Source: CAD feature listing. Evaluate the final solid. Frame: model axes, mm. A direction names the side the tool comes from. Coordinates: 2 decimals unless noted, no trailing zeros. Write each loop counter-clockwise with the first axis right and the second up, starting at its lowest first coordinate (ties: lowest second). Pieces come first, ordered by that corner, then holes. Notation, with made-up numbers: (-32.75, 44.5) - (16.25, 44.5) arc R22 cw to (16.25, 67.5) - close; hole circle Ø1 at (20.25, -19). An arc over 180 degrees is marked (long way). One line per item, written item: value.
from build123d import *

# Parameters (mm, degrees)
EXTRUDE_1_DEPTH     = 15
SKETCH_2_R          = 13
CUT_EXTRUDE_2_DEPTH = 10


with BuildPart() as part:
    # 草图1 → 拉伸1 (new, symmetric)
    with BuildSketch(Plane.XY):
        with BuildLine():
            ThreePointArc((-7.220859013, 49.475844562), (-35.355230678, 35.355447441), (-49.47580029, 7.221162349))
            add(Edge.make_bspline(
                [(-49.47580029, -7.221162349), (-36.725591286, 0), (-49.47580029, 7.221162349)],
                knots=[2.665650331, 2.665650331, 2.665650331, 3.617534976, 3.617534976, 3.617534976], degree=2, weights=[1, 0.888861367, 1]))
            ThreePointArc((-49.47580029, -7.221162349), (-35.355230678, -35.355447441), (-7.220859013, -49.475844562))
            add(Edge.make_bspline(
                [(7.220859013, -49.475844562), (0, -36.72563521), (-7.220859013, -49.475844562)],
                knots=[2.665650231, 2.665650231, 2.665650231, 3.617535076, 3.617535076, 3.617535076], degree=2, weights=[1, 0.888861321, 1]))
            ThreePointArc((7.220859013, -49.475844562), (35.063945901, -35.644350154), (49.350641932, -8.032069525))
            add(Edge.make_bspline(
                [(49.350641932, 8.032069525), (36.37710154, 0), (49.350641932, -8.032069525)],
                knots=[5.748433423, 5.748433423, 5.748433423, 6.817937192, 6.817937192, 6.817937192], degree=2, weights=[1, 0.860395102, 1]))
            ThreePointArc((49.350641932, 8.032069525), (35.063945901, 35.644350154), (7.220859013, 49.475844562))
            add(Edge.make_bspline(
                [(-7.220859013, 49.475844562), (0, 36.72563521), (7.220859013, 49.475844562)],
                knots=[2.665650231, 2.665650231, 2.665650231, 3.617535076, 3.617535076, 3.617535076], degree=2, weights=[1, 0.888861321, 1]))
        make_face()
        with BuildLine():
            Line((3, -6.873863542), (3, -12.5))
            Line((3, -12.5), (-3, -12.5))
            Line((-3, -12.5), (-3, -6.873863542))
            ThreePointArc((-3, -6.873863542), (-5.303300859, -5.303300859), (-6.873863542, -3))
            Line((-6.873863542, -3), (-12.5, -3))
            Line((-12.5, -3), (-12.5, 3))
            Line((-12.5, 3), (-6.873863542, 3))
            ThreePointArc((-6.873863542, 3), (-5.303300859, 5.303300859), (-3, 6.873863542))
            Line((-3, 6.873863542), (-3, 12.5))
            Line((-3, 12.5), (3, 12.5))
            Line((3, 12.5), (3, 6.873863542))
            ThreePointArc((3, 6.873863542), (5.303300859, 5.303300859), (6.873863542, 3))
            Line((6.873863542, 3), (12.5, 3))
            Line((12.5, 3), (12.5, -3))
            Line((12.5, -3), (6.873863542, -3))
            ThreePointArc((6.873863542, -3), (5.303300859, -5.303300859), (3, -6.873863542))
        make_face(mode=Mode.SUBTRACT)
    extrude(amount=EXTRUDE_1_DEPTH, both=True)

    # 草图2 → 拉伸2 (cut)
    with BuildSketch(Plane.XY.offset(15)):
        Circle(SKETCH_2_R)
    extrude(amount=-CUT_EXTRUDE_2_DEPTH, mode=Mode.SUBTRACT)


solid = part.part
1) Section query A-A on y = 15. Output: boundary loops of the cut face in (x, z), then the cut area to 3 significant figures.
Values found:
outline: (-47.7, -15) - (47.7, -15) - (47.7, 15) - (-47.7, 15) - close
area: 2,860 mm2
2) Material intervals for line 1 (Y direction, x = 0, z = 10.75); line 2 (X direction, y = 12, z = -4.5); line 3 (X direction, y = 8, z = -13), sorted ascending.
Values found:
line 1: -43.48 to -13, 13 to 43.48
line 2: -48.54 to -3, 3 to 48.54
line 3: -49.36 to -3, 3 to 49.3
3) Contact query for flat-ended pins moving along their axis: P1, Ø21, axis at x = 1, y = 1, coming from the +Z side; P2, Ø3, axis at y = 0, z = -9.5, coming from the +X side; P3, Ø1.5, axis at x = -12, z = 8, coming from the +Y side. Output: stop coordinate, or through.
Values found:
P1: z = 5
P2: x = 43.55
P3: y = 48.72
4) Reachability of faces 1 (the cylindrical face through (-10.316, -7.91, 10.07)), 2 (the flat face through (10, -10, -15)), 3 (the flat face through (3, 10, -5)) from +Z, -Z, +X, -X, +Y, -Y: full face, straight path, thin tool, end or side. Return the list, or none.
Values found:
face 1: +Z
face 2: -Z, +X, -X, +Y, -Y
face 3: +Z, -Z
5) Draft query along Y for faces 4 (the cylindrical face through (34.7, -36, 0.2)), 5 (the cylindrical face through (-35.04, 35.67, 0.21)), 6 (the cylindrical face through (-5.275, -5.331, -4.86)), 7 (the flat face through (-5, 6, 5)). Return one class per face: released by +Y, released by -Y, zero draft, split by the parting line, or undercut.
Values found:
face 4: released by -Y
face 5: released by +Y
face 6: undercut
face 7: undercut
6) Section query B-B on x = -20. Output: boundary loops of the cut face in (y, z), then the cut area to 3 significant figures.
Values found:
outline: (-45.83, -15) - (45.83, -15) - (45.83, 15) - (-45.83, 15) - close
area: 2,750 mm2
